from build123d import *

# Parameters (mm, degrees)
SKETCH_1_W                = 150
SKETCH_1_H                = 450
EXTRUDE_1_DEPTH           = 30
SKETCH_2_W                = 28.5
SKETCH_2_H                = 450
CUT_EXTRUDE_1_DEPTH       = 5
HOLE_WIZARD_M8_1_D        = 6.8
PATTERN_LINEAR_1_COUNT    = 5
PATTERN_LINEAR_1_PITCH    = 80
HOLE_WIZARD_1_D           = 9
HOLE_WIZARD_1_CBORE_D     = 15
HOLE_WIZARD_1_CBORE_DEPTH = 9
PATTERN_LINEAR_2_COUNT    = 5
PATTERN_LINEAR_2_PITCH    = 80
SKETCH_7_W                = 56.5
SKETCH_7_H                = 450
CUT_EXTRUDE_2_DEPTH       = 15
HOLE_WIZARD_2_D           = 9
HOLE_WIZARD_2_CBORE_D     = 15
HOLE_WIZARD_2_CBORE_DEPTH = 9


with BuildPart() as part:
    # 草图1 → 凸台-拉伸1 (new body)
    with BuildSketch(Plane(origin=(0, 0, 0), x_dir=(0, 0, -1), z_dir=(1, 0, 0))):
        Rectangle(SKETCH_1_W, SKETCH_1_H)
    extrude(amount=EXTRUDE_1_DEPTH)

    # 草图2 → 切除-拉伸1 (cut)
    with BuildSketch(Plane(origin=(30, 0, 0), x_dir=(0, 0, -1), z_dir=(1, 0, 0))):
        with Locations((-42.5, 0)):
            Rectangle(SKETCH_2_W, SKETCH_2_H)
        with Locations((42.5, 0)):
            Rectangle(SKETCH_2_W, SKETCH_2_H)
    extrude(amount=-CUT_EXTRUDE_1_DEPTH, mode=Mode.SUBTRACT)

    # M8 螺纹孔1 (through all)
    with Locations(Plane(origin=(30, 0, 0), x_dir=(0, 0, -1), z_dir=(1, 0, 0))):
        with Locations((-42.5, -155), (42.5, -155)):
            hole_wizard_m8_1 = Hole(HOLE_WIZARD_M8_1_D / 2)

    # 阵列(线性)1: M8 螺纹孔1 ×5
    with Locations(*[(0, i * PATTERN_LINEAR_1_PITCH, 0) for i in range(1, PATTERN_LINEAR_1_COUNT)]):
        add(hole_wizard_m8_1, mode=Mode.SUBTRACT)

    # 打孔尺寸(%根据)内六角圆柱头螺钉的类型1 (through all)
    with Locations(Plane(origin=(25, 0, 0), x_dir=(0, 0, -1), z_dir=(1, 0, 0))):
        with Locations((-42.5, -115), (42.5, -115)):
            hole_wizard_1 = CounterBoreHole(HOLE_WIZARD_1_D / 2, HOLE_WIZARD_1_CBORE_D / 2, HOLE_WIZARD_1_CBORE_DEPTH)

    # 阵列(线性)2: 打孔尺寸(%根据)内六角圆柱头螺钉的类型1 ×5
    with Locations(*[(0, i * PATTERN_LINEAR_2_PITCH, 0) for i in range(1, PATTERN_LINEAR_2_COUNT)]):
        add(hole_wizard_1, mode=Mode.SUBTRACT)

    # 草图7 → 切除-拉伸2 (cut)
    with BuildSketch(Plane(origin=(30, 0, 0), x_dir=(0, 0, -1), z_dir=(1, 0, 0))):
        Rectangle(SKETCH_7_W, SKETCH_7_H)
    extrude(amount=-CUT_EXTRUDE_2_DEPTH, mode=Mode.SUBTRACT)

    # 打孔尺寸(%根据)内六角圆柱头螺钉的类型2 (through all)
    with Locations(Plane(origin=(0, 0, 0), x_dir=(0, 0, -1), z_dir=(-1, 0, 0))):
        with Locations((-12.5, 185.5), (12.5, 185.5), (-12.5, 215.5), (12.5, 215.5)):
            CounterBoreHole(HOLE_WIZARD_2_D / 2, HOLE_WIZARD_2_CBORE_D / 2, HOLE_WIZARD_2_CBORE_DEPTH)


solid = part.part
The listing builds one solid part. Answer for the finished solid, in the listing's coordinates (mm). A direction names the side the tool comes from. Coordinates: 2 decimals unless noted, no trailing zeros. Loops run counter-clockwise (first coordinate to the right, second up) from the corner with the lowest first, then second, coordinate; pieces in that order, holes last.
1) Find section A-A on y = -215.5. Write down the section's boundary in (x, z), then the cut area to 3 significant figures.
2) Flat-ended cylindrical pins translate along their axes: pin 1 Ø5 at (y, z) = (6, -46) entering from +X; pin 2 Ø7 at (y, z) = (-215.5, -12.5) entering from -X; pin 3 Ø12 at (y, z) = (-185.5, -12.5) entering from -X; pin 4 Ø12 at (y, z) = (-185.5, 12.5) entering from +X. Find the tip coordinate at first contact, or state that the pin passes through.
3) Find section B-B on y = 205. Write down the section's boundary in (x, z), then the cut area to 3 significant figures.
4) A tool of negligible diameter and unlimited length cuts with its end or side. For faces 4 (the face through (9, -182, 9)), 5 (the face through (20.563, 212.436, -41.524)), 6 (the face through (7.89, 200.61, -43.48)), 7 (the face through (25, 3, 46)), from which of +Z, -Z, +X, -X, +Y, -Y can it reach the whole face along a straight path? Write none if from no direction.
5) Determine the mould class of faces 1 (the face through (11, -225, 1)), 2 (the face through (7.89, 200.61, 41.52)), 3 (the face through (15, -3, -75)) for opening direction Z: pulls with the +Z half, pulls with the -Z half, needs draft (parallel to the pull), parting line crosses it, or undercut.
6) Find the intervals of material crossed by L1, parallel to Z at x = 3.25, y = 122; L2, parallel to Y at x = 11.25, z = 12.5; L3, parallel to Y at x = 2.5, z = 12.5, in increasing order.
7) Find section C-C on y = 155.5. Write down the section's boundary in (x, z), then the cut area to 3 significant figures.
Values:
1. outline: (0, -75) - (30, -75) - (30, -56.75) - (25, -56.75) - (25, -28.25) - (15, -28.25) - (15, -17) - (9, -17) - (9, -20) - (0, -20) - close; (0, -5) - (9, -5) - (9, -8) - (15, -8) - (15, 8) - (9, 8) - (9, 5) - (0, 5) - close; (0, 20) - (9, 20) - (9, 17) - (15, 17) - (15, 28.25) - (25, 28.25) - (25, 56.75) - (30, 56.75) - (30, 75) - (0, 75) - close
1. area: 2,990 mm2
2. pin 1: stops at x = 25
2. pin 2: passes through
2. pin 3: stops at x = 9
2. pin 4: stops at x = 15
3. outline: (0, -75) - (30, -75) - (30, -56.75) - (25, -56.75) - (25, -50) - (16, -50) - (16, -47) - (0, -47) - close; (0, -38) - (16, -38) - (16, -35) - (25, -35) - (25, -28.25) - (15, -28.25) - (15, 28.25) - (25, 28.25) - (25, 35) - (16, 35) - (16, 38) - (0, 38) - close; (0, 47) - (16, 47) - (16, 50) - (25, 50) - (25, 56.75) - (30, 56.75) - (30, 75) - (0, 75) - close
3. area: 2,810 mm2
4. face 4: -X
4. face 5: +X
4. face 6: +X, -X
4. face 7: +X, +Y, -Y
5. face 1: needs draft
5. face 2: undercut
5. face 3: pulls with the -Z half
6. L1: z = -75 to -45.85, -39.15 to 39.15, 45.85 to 75
6. L2: y = -225 to -220, -211 to -190, -181 to 225
6. L3: y = -225 to -223, -208 to -193, -178 to 225
7. outline: (0, -75) - (30, -75) - (30, -56.75) - (25, -56.75) - (25, -28.25) - (15, -28.25) - (15, 28.25) - (25, 28.25) - (25, 56.75) - (30, 56.75) - (30, 75) - (0, 75) - close
7. area: 3,370 mm2
